Verification items for the finished model (mm, model axes). Round coordinates to 2 decimals unless told otherwise and drop trailing zeros. Order: outer loops, then holes, each group sorted by start corner. A loop starts at its lowest first (then second) coordinate and runs counter-clockwise, first axis right, second up. Notation, with made-up numbers: M 26.25,45 L 48.25,45 A31 cw 48.25,80 Z; hole C 3,79 d11. An arc over 180 degrees is marked long. Write item = value, one per line. Start each with the question number.
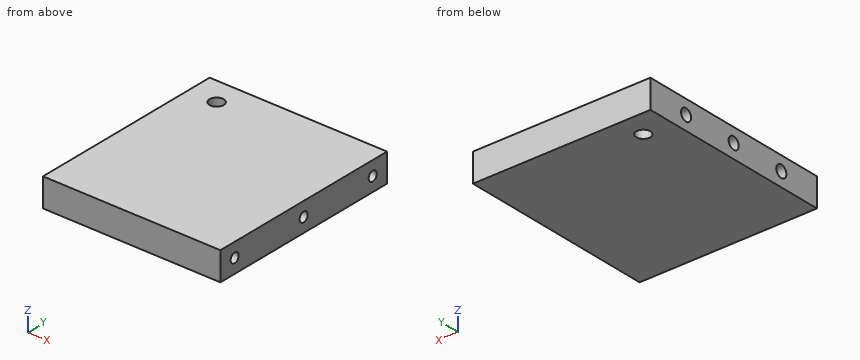
from build123d import *

# Parameters (mm, degrees)
SKETCH1_W              = 125
SKETCH1_H              = 140
BOSS_EXTRUDE1_DEPTH    = 20
M10_TAPPED_HOLE1_D     = 8.5
M10_TAPPED_HOLE1_DEPTH = 35
M10_TAPPED_HOLE1_TIP   = 2.553657631
M8_TAPPED_HOLE1_D      = 6.8
M8_TAPPED_HOLE1_DEPTH  = 22.25
M8_TAPPED_HOLE1_TIP    = 2.042926105
SKETCH6_R              = 5
CUT_EXTRUDE1_DEPTH     = 96.949205312


with BuildPart() as part:
    # Sketch1 → Boss-Extrude1 (new body)
    with BuildSketch(Plane.XY):
        Rectangle(SKETCH1_W, SKETCH1_H)
    extrude(amount=BOSS_EXTRUDE1_DEPTH)

    # M10 Tapped Hole1
    with Locations(Plane.ZY.offset(62.5)):
        with Locations((10, 40), (10, 0), (10, -40)):
            Hole(M10_TAPPED_HOLE1_D / 2, depth=M10_TAPPED_HOLE1_DEPTH)
            with Locations((0, 0, -(M10_TAPPED_HOLE1_DEPTH + M10_TAPPED_HOLE1_TIP / 2))):  # 118° drill point
                Cone(0, M10_TAPPED_HOLE1_D / 2, M10_TAPPED_HOLE1_TIP, mode=Mode.SUBTRACT)

    # M8 Tapped Hole1
    with Locations(Plane(origin=(62.5, 0, 0), x_dir=(0, 0, -1), z_dir=(1, 0, 0))):
        with Locations((-10, 58), (-10, 0), (-10, -58)):
            Hole(M8_TAPPED_HOLE1_D / 2, depth=M8_TAPPED_HOLE1_DEPTH)
            with Locations((0, 0, -(M8_TAPPED_HOLE1_DEPTH + M8_TAPPED_HOLE1_TIP / 2))):  # 118° drill point
                Cone(0, M8_TAPPED_HOLE1_D / 2, M8_TAPPED_HOLE1_TIP, mode=Mode.SUBTRACT)

    # Sketch6 → Cut-Extrude1 (cut, through all)
    with BuildSketch(Plane.XY.offset(20)):
        with Locations((-42.5, 52)):
            Circle(SKETCH6_R)
    extrude(amount=-CUT_EXTRUDE1_DEPTH, mode=Mode.SUBTRACT)


solid = part.part
1) Scan lines: probe 1 along Y at (x, z) = (53, 10); probe 2 along Y at (x, z) = (-54, 10); probe 3 along Z at (x, y) = (-27, 40.5). Record each from-to range of solid material in increasing order.
2) Gauge pin test, flat ends, axial feed: P1, Ø7, axis at y = 40, z = 10, coming from the -X side; P2, Ø6, axis at y = -58, z = 10, coming from the +X side; P3, Ø4, axis at y = 0, z = 10, coming from the -X side. Record the tip position at first contact, or that the pin passes through.
3) Cross-section at A-A, the plane x = 42. Enter the section's corners in (y, z), then the cut area to 3 significant figures.
Geometry results:
q1.probe_1 = -70 to -61.4, -54.6 to -3.4, 3.4 to 54.6, 61.4 to 70
q1.probe_2 = -70 to -44.25, -35.75 to -4.25, 4.25 to 35.75, 44.25 to 70
q1.probe_3 = 0 to 6.62, 13.38 to 20
q2.P1 = -27.05
q2.P2 = 40.01
q2.P3 = -26.15
q3.outline = M -70,0 L 70,0 L 70,20 L -70,20 Z; hole C -58,10 d6.8; hole C 0,10 d6.8; hole C 58,10 d6.8
q3.area = 2,690 mm^2
